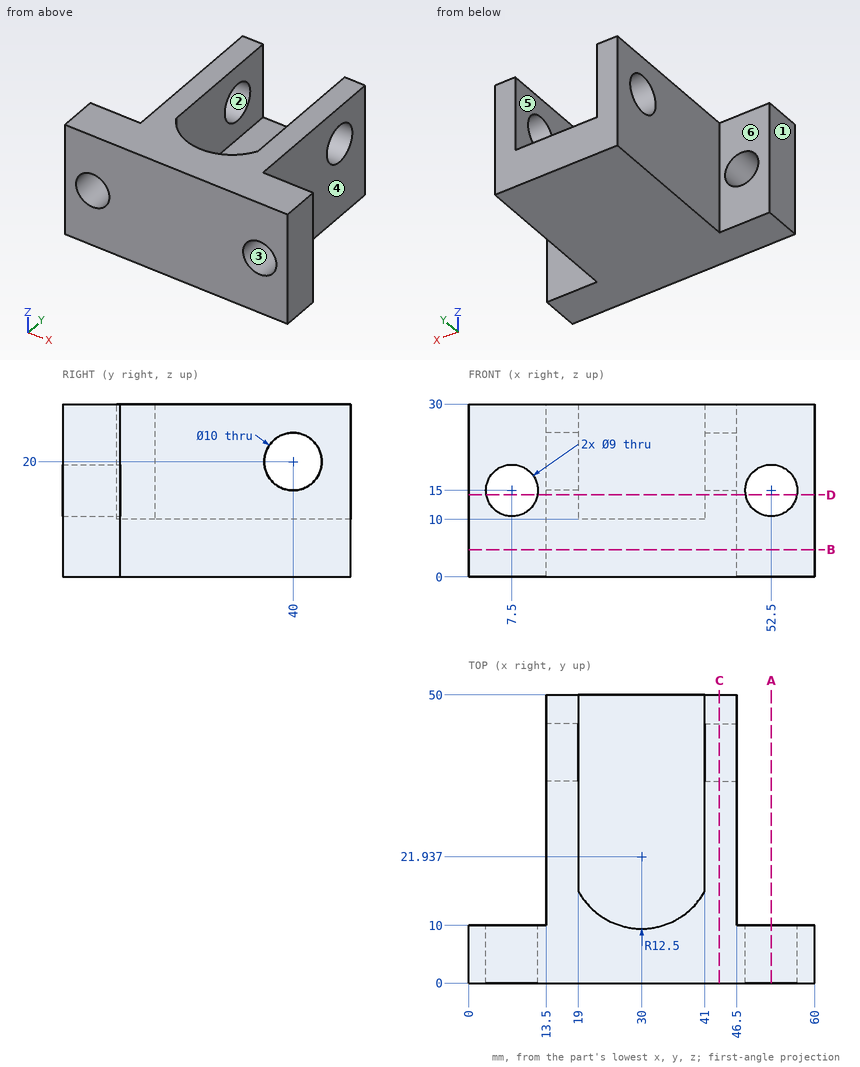
Study the drawing (mm; zero at the part's minimum x, y, z) and answer. A direction names the side the tool comes from. Coordinates: 2 decimals unless noted, no trailing zeros. Loops run counter-clockwise (first coordinate to the right, second up) from the corner with the lowest first, then second, coordinate; pieces in that order, holes last. Notation, with made-up numbers: M 40,12.5 L 51,12.5 A10 ccw 51,17.5 Z; hole C 27,40.25 d11. An arc over 180 degrees is marked long. Answer in a Markdown table with one row per item. Add a question column.
1. Find section A-A, the plane x = 52.5. Write down the section's boundary in (y, z), then the cut area to 3 significant figures.
2. Find section C-C, the plane x = 43.5. Write down the section's boundary in (y, z).
3. Consider L1, parallel to Y at x = 14.5, z = 20; L2, parallel to X at y = 48, z = 28.25; L3, parallel to Z at x = 52.5, y = 7.25. Determine where each line is inside the solid, lowest interval first.
4. Find section B-B, the plane z = 4.75. Write down the section's boundary in (x, y).
5. Flat-ended cylindrical pins translate along their axes: P1, Ø10, axis at y = 31.5, z = 22.5, coming from the +X side; P2, Ø3, axis at y = 24.5, z = 8, coming from the -X side; P3, Ø11, axis at x = 8.5, z = 20, coming from the +Y side; P4, Ø6.5, axis at x = 28.5, y = 31, coming from the +Z side. Find the tip coordinate at first contact, or state that the pin passes through.
6. Find section D-D, the plane z = 14.25. Write down the section's boundary in (x, y), then the cut area to 3 significant figures.
7. The mould has two halves that part along X. Classify the marked faces 1, 2 and 3: pulls with the +X half, pulls with the -X half, needs draft (parallel to the pull), parting line crosses it, or undercut.
8. A tool of negligible diameter and unlimited length cuts with its end or side. For the marked faces 4, 5 and 6, from which of +Z, -Z, +X, -X, +Y, -Y can it reach the whole face along a straight path? Write none if from no direction.
Reported:
| question | item | result |
|---|---|---|
| 1 | outline | M 0,0 L 10,0 L 10,10.5 L 0,10.5 Z; M 0,19.5 L 10,19.5 L 10,30 L 0,30 Z |
| 1 | area | 210 mm^2 |
| 2 | outline | M 0,0 L 50,0 L 50,30 L 0,30 Z; hole C 40,20 d10 |
| 3 | L1 | y = 0 to 35, 45 to 50 |
| 3 | L2 | x = 13.5 to 19, 41 to 46.5 |
| 3 | L3 | z = 0 to 10.5, 19.5 to 30 |
| 4 | outline | M 0,0 L 60,0 L 60,10 L 46.5,10 L 46.5,50 L 13.5,50 L 13.5,10 L 0,10 Z |
| 5 | P1 | stops at x = 46.5 |
| 5 | P2 | stops at x = 13.5 |
| 5 | P3 | stops at y = 50 |
| 5 | P4 | stops at z = 10 |
| 6 | outline | M 0,0 L 3.06,0 L 3.06,10 L 0,10 Z; M 11.94,0 L 48.06,0 L 48.06,10 L 46.5,10 L 46.5,50 L 41,50 L 41,16 A12.5 cw 19,16 L 19,50 L 13.5,50 L 13.5,10 L 11.94,10 Z; M 56.94,0 L 60,0 L 60,10 L 56.94,10 Z |
| 6 | area | 892 mm^2 |
| 7 | face 1 | pulls with the -X half |
| 7 | face 2 | needs draft |
| 7 | face 3 | undercut |
| 8 | face 4 | +Z, -Z, +X, +Y |
| 8 | face 5 | +Z, +Y |
| 8 | face 6 | +Z, -Z, -X, +Y |
